from build123d import *

# Parameters (mm, degrees)
BOSS_EXTRUDE1_DEPTH = 8
CHAMFER1_SIZE       = 15


with BuildPart() as part:
    # Sketch1 → Boss-Extrude1 (new body)
    with BuildSketch(Plane.XY):
        Polygon((0, 0), (50, 0), (50, 15), (15, 110), (0, 110), align=None)
    extrude(amount=BOSS_EXTRUDE1_DEPTH)

    # Chamfer1
    chamfer1_edges = [part.edges().sort_by_distance(p)[0] for p in [
        (0, 0, 4),
    ]]
    chamfer(chamfer1_edges, length=CHAMFER1_SIZE)


solid = part.part
The model under review builds one solid part; all positions refer to its coordinate system, in mm. Round coordinates to 2 decimals unless told otherwise and drop trailing zeros. Write each loop counter-clockwise with the first axis right and the second up, starting at its lowest first coordinate (ties: lowest second). Pieces come first, ordered by that corner, then holes. Notation, with made-up numbers: M 40.25,65.5 L 91.25,65.5 A19 cw 91.25,78.5 Z; hole C 9.25,24 d1. An arc over 180 degrees is marked long. Answer as CSV lines item,"result". Start each with the question number.
Q1. Consider section C-C, the plane x = 8.5. Give the boundary of the cut face in (y, z), then the cut area to 3 significant figures.
Q2. Consider section B-B, the plane y = 13. Give the boundary of the cut face in (x, z).
Q3. Clearance check with a flat-ended pin moving along its axis: P1, Ø8, axis at x = 33, y = 75.5, coming from the +Z side. State where the tip first meets the part, or that it passes through.
Q4. Wall thickness on line 1 along Y through (x, z) = (7, 0.5); line 2 along X through (y, z) = (100, 1.75); line 3 along X through (y, z) = (17, 1.75): over which ranges is each line inside the solid? List them lowest first.
Q5. Consider section A-A, the plane z = 6.5. Give the boundary of the cut face in (x, y), then the cut area to 4 significant figures.
Q6. The part is to be moulded in two halves that separate along X. For faces 1 (the face through (0, 63, 4)), 2 (the face through (50, 7, 4)), 3 (the face through (19, 44, 8)), say which applies: +X half, -X half, draft (parallel to the pull), parting line (faces both ways), or undercut.
Result set:
1,outline,"M 6.5,0 L 110,0 L 110,8 L 6.5,8 Z"
1,area,"828 mm²"
2,outline,"M 2,0 L 50,0 L 50,8 L 2,8 Z"
3,P1,"passes through"
4,line 1,"y = 8 to 110"
4,line 2,"x = 0 to 18.68"
4,line 3,"x = 0 to 49.26"
5,outline,"M 0,15 L 15,0 L 50,0 L 50,15 L 15,110 L 0,110 Z"
5,area,"3,725 mm²"
6,face 1,"-X half"
6,face 2,"+X half"
6,face 3,"draft"
